Read the model definition and answer for the solid it produces. Units are mm, in the model's axes. Face numbers are marked on the shaded views. A direction names the side the tool comes from. Coordinates: 2 decimals unless noted, no trailing zeros. Write each loop counter-clockwise with the first axis right and the second up, starting at its lowest first coordinate (ties: lowest second). Pieces come first, ordered by that corner, then holes. Notation, with made-up numbers: (7, 65) -> (39, 65) arc R16 cw to (39, 86) -> close; hole circle Ø8 at (1, 31.25). An arc over 180 degrees is marked (long way). One line per item, written item: value. Start each with the question number.
1. Given P1, Ø8, axis at y = 47.5, z = 9.5, coming from the +X side; P2, Ø12, axis at x = -2, y = -21.5, coming from the -Z side; P3, Ø12, axis at x = -2.5, z = 44, coming from the -Y side, each flat-ended and moving along its own axis, determine where each tip first touches the part or whether it passes through.
2. Find section A-A, the plane z = 9.5. Write down the section's boundary in (x, y).
3. Find section D-D, the plane z = 72. Write down the section's boundary in (x, y).
4. For the marked faces 1 and 2, determine the directions among +Z, -Z, +X, -X, +Y, -Y from which every point of the face is accessible in a straight line to the end or side of a thin tool.
5. Find section C-C, the plane x = 1. Write down the section's boundary in (y, z).
6. Find section B-B, the plane y = 47.5. Write down the section's boundary in (x, z), and give its area (3 significant figures).
7. Consider line 1 along X through (y, z) = (24.5, 39.5); line 2 along Y through (x, z) = (-46.3, 9.5); line 3 along Y through (x, z) = (-46.05, 9.5). Determine where each line is inside the solid, lowest interval first.
8. For a pull along X with two mould halves and no side action, classify the marked faces 3, 4, 5 and 6 as pulls with the +X half, pulls with the -X half, needs draft (parallel to the pull), parting line crosses it, or undercut.
```python
from build123d import *

# Parameters (mm, degrees)
SKETCH_1_W          = 93.5
SKETCH_1_H          = 123
SKETCH_1_W_2        = 90.5
SKETCH_1_H_2        = 120
EXTRUDE_1_DEPTH     = 100
SKETCH_2_W          = 93.5
SKETCH_2_H          = 123
EXTRUDE_2_DEPTH     = 1.5
SKETCH_3_W          = 90.5
SKETCH_3_H          = 98.5
CUT_EXTRUDE_1_DEPTH = 3
SKETCH_4_R          = 3.5
CUT_EXTRUDE_2_DEPTH = 151.081644447
FILLET_1_R          = 2
FILLET_2_R          = 3.5
FILLET_3_R          = 1
FILLET_4_R          = 1.5


with BuildPart() as part:
    # 草图1 → 凸台-拉伸1 (new body)
    with BuildSketch(Plane.XY):
        Rectangle(SKETCH_1_W, SKETCH_1_H)
        Rectangle(SKETCH_1_W_2, SKETCH_1_H_2, mode=Mode.SUBTRACT)
    extrude(amount=EXTRUDE_1_DEPTH)

    # 草图2 → 凸台-拉伸2 (add)
    with BuildSketch(Plane.XY.offset(100)):
        Rectangle(SKETCH_2_W, SKETCH_2_H)
    extrude(amount=-EXTRUDE_2_DEPTH)

    # 草图3 → 切除-拉伸1 (cut)
    with BuildSketch(Plane.XZ.offset(61.5)):
        with Locations((0, 49.25)):
            Rectangle(SKETCH_3_W, SKETCH_3_H)
    extrude(amount=-CUT_EXTRUDE_1_DEPTH, mode=Mode.SUBTRACT)

    # 草图4 → 切除-拉伸2 (cut, through all)
    with BuildSketch(Plane(origin=(46.75, 0, 0), x_dir=(0, 0, -1), z_dir=(1, 0, 0))):
        with Locations((-9.5, -44.5)):
            Circle(SKETCH_4_R)
        with Locations((-9.5, 47.5)):
            Circle(SKETCH_4_R)
    extrude(amount=-CUT_EXTRUDE_2_DEPTH, mode=Mode.SUBTRACT)

    # 圆角1
    fillet_1_edges = [part.edges().sort_by_distance(p)[0] for p in [
        (45.25, -0.75, 98.5),
        (-45.25, -0.75, 98.5),
    ]]
    fillet(fillet_1_edges, radius=FILLET_1_R)

    # 圆角2
    fillet_2_edges = [part.edges().sort_by_distance(p)[0] for p in [
        (-46.75, 0, 100),
        (46.75, 0, 100),
    ]]
    fillet(fillet_2_edges, radius=FILLET_2_R)

    # 圆角3
    fillet_3_edges = [part.edges().sort_by_distance(p)[0] for p in [
        (-45.25, 60, 48.25),
        (0, 60, 98.5),
        (45.25, 60, 48.25),
        (44.664213562, 60, 97.914213562),
        (-44.664213562, 60, 97.914213562),
    ]]
    fillet(fillet_3_edges, radius=FILLET_3_R)

    # 圆角4
    fillet_4_edges = [part.edges().sort_by_distance(p)[0] for p in [
        (46.75, 61.5, 48.25),
        (-46.75, 61.5, 48.25),
        (-45.724873734, 61.5, 98.974873734),
        (45.724873734, 61.5, 98.974873734),
        (0, 61.5, 100),
    ]]
    fillet(fillet_4_edges, radius=FILLET_4_R)


solid = part.part
```
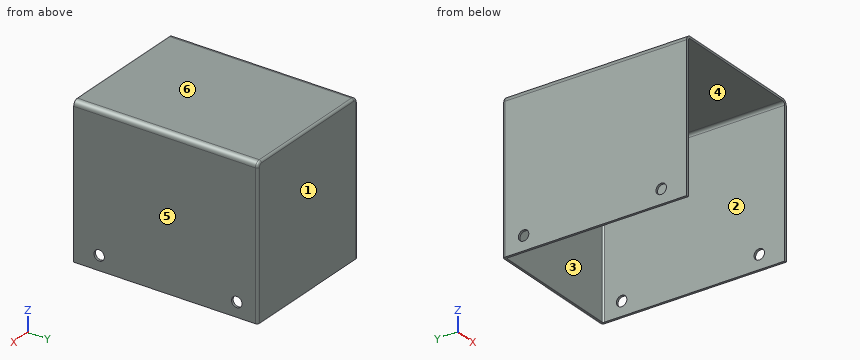
Answer block:
1. P1: stops at x = 46.75
1. P2: stops at z = 98.5
1. P3: stops at y = 60
2. outline: (-46.75, -61.5) -> (-45.25, -61.5) -> (-45.25, -48) -> (-46.75, -48) -> close; (-46.75, -41) -> (-45.25, -41) -> (-45.25, 44) -> (-46.75, 44) -> close; (-46.75, 51) -> (-45.25, 51) -> (-45.25, 59) arc R1 cw to (-44.25, 60) -> (44.25, 60) arc R1 cw to (45.25, 59) -> (45.25, 51) -> (46.75, 51) -> (46.75, 60) arc R1.5 ccw to (45.25, 61.5) -> (-45.25, 61.5) arc R1.5 ccw to (-46.75, 60) -> close; (45.25, -61.5) -> (46.75, -61.5) -> (46.75, -48) -> (45.25, -48) -> close; (45.25, -41) -> (46.75, -41) -> (46.75, 44) -> (45.25, 44) -> close
3. outline: (-46.75, -61.5) -> (-45.25, -61.5) -> (-45.25, 59) arc R1 cw to (-44.25, 60) -> (44.25, 60) arc R1 cw to (45.25, 59) -> (45.25, -61.5) -> (46.75, -61.5) -> (46.75, 60) arc R1.5 ccw to (45.25, 61.5) -> (-45.25, 61.5) arc R1.5 ccw to (-46.75, 60) -> close
4. face 1: +Z, -Z, +X, -X, +Y
4. face 2: -Z, -Y
5. outline: (-61.5, 98.5) -> (59, 98.5) arc R1 cw to (60, 97.5) -> (60, 0) -> (61.5, 0) -> (61.5, 98.5) arc R1.5 ccw to (60, 100) -> (-61.5, 100) -> close
6. outline: (-46.75, 0) -> (-45.25, 0) -> (-45.25, 6) -> (-46.75, 6) -> close; (-46.75, 13) -> (-45.25, 13) -> (-45.25, 96.5) arc R2 cw to (-43.25, 98.5) -> (43.25, 98.5) arc R2 cw to (45.25, 96.5) -> (45.25, 13) -> (46.75, 13) -> (46.75, 96.5) arc R3.5 ccw to (43.25, 100) -> (-43.25, 100) arc R3.5 ccw to (-46.75, 96.5) -> close; (45.25, 0) -> (46.75, 0) -> (46.75, 6) -> (45.25, 6) -> close
6. area: 411 mm2
7. line 1: x = -46.75 to -45.25, 45.25 to 46.75
7. line 2: y = -61.5 to -48, -41 to 44, 51 to 61.07
7. line 3: y = -61.5 to -48, -41 to 44, 51 to 61.27
8. face 3: undercut
8. face 4: undercut
8. face 5: pulls with the +X half
8. face 6: needs draft
